Geometry check sheet. Reference: the model listing, model coordinates, mm. A direction names the side the tool comes from. Coordinates: 2 decimals unless noted, no trailing zeros. Loops run counter-clockwise (first coordinate to the right, second up) from the corner with the lowest first, then second, coordinate; pieces in that order, holes last.
from build123d import *

# Parameters (mm, degrees)
SKETCH1_W           = 65
SKETCH1_H           = 30
BOSS_EXTRUDE1_DEPTH = 950
SKETCH2_W           = 59
SKETCH2_H           = 24
CUT_EXTRUDE1_DEPTH  = 950
SKETCH5_R           = 4
CUT_EXTRUDE2_DEPTH  = 954.05282071


with BuildPart() as part:
    # Sketch1 → Boss-Extrude1 (new body)
    with BuildSketch(Plane.XY):
        with Locations((-8.040751589, 24.808027615)):
            Rectangle(SKETCH1_W, SKETCH1_H)
    extrude(amount=BOSS_EXTRUDE1_DEPTH)

    # Sketch2 → Cut-Extrude1 (cut)
    with BuildSketch(Plane.XY.offset(950)):
        with Locations((-8.040751589, 24.808027615)):
            Rectangle(SKETCH2_W, SKETCH2_H)
    extrude(amount=-CUT_EXTRUDE1_DEPTH, mode=Mode.SUBTRACT)

    # Sketch5 → Cut-Extrude2 (cut, through all)
    with BuildSketch(Plane.ZY.offset(40.540751589)):
        with Locations((445.101574912, 26.308027615)):
            Circle(SKETCH5_R)
        with Locations((613.101574912, 26.308027615)):
            Circle(SKETCH5_R)
        with Locations((757.101574912, 26.308027615)):
            Circle(SKETCH5_R)
    extrude(amount=-CUT_EXTRUDE2_DEPTH, mode=Mode.SUBTRACT)


solid = part.part
(1) Access from +Z, -Z, +X, -X, +Y, -Y to the whole of each face (thin tool, end or side, straight path). Record for faces 1 (the flat face through (-8, 36.808, 482)), 2 (the flat face through (-40.541, 25, 468)).
Findings:
face 1: +Z, -Z
face 2: +Z, -Z, -X, +Y, -Y
(2) Scan lines: L1, parallel to X at y = 14.25, z = 102; L2, parallel to Y at x = -22.5, z = 767.5. Record each from-to range of solid material in increasing order.
Findings:
L1: x = -40.54 to -37.54, 21.46 to 24.46
L2: y = 9.81 to 12.81, 36.81 to 39.81
(3) Sectioned sample at A-A on x = 9.5. Record the cut outline in (y, z).
Findings:
outline: (9.81, 0) - (12.81, 0) - (12.81, 950) - (9.81, 950) - close; (36.81, 0) - (39.81, 0) - (39.81, 950) - (36.81, 950) - close
(4) Sectioned sample at B-B on z = 268. Record the cut outline in (x, y), and give its area (3 significant figures).
Findings:
outline: (-40.54, 9.81) - (24.46, 9.81) - (24.46, 39.81) - (-40.54, 39.81) - close; hole (-37.54, 12.81) - (21.46, 12.81) - (21.46, 36.81) - (-37.54, 36.81) - close
area: 534 mm2
(5) Draft check along Y on faces 3 (the flat face through (-8, 12.808, 482)), 4 (the flat face through (-8, 39.808, 468)), 5 (the flat face through (-37.541, 25, 482)), 6 (the flat face through (-8, 9.808, 468)). Enter one of: +Y half, -Y half, draft (parallel to the pull), parting line (faces both ways), or undercut.
Findings:
face 3: undercut
face 4: +Y half
face 5: undercut
face 6: -Y half
